The listing builds one solid part. Answer for the finished solid, in the listing's coordinates (mm). Face numbers are marked on the shaded views. A direction names the side the tool comes from. Give positions to 0.01 mm unless a question says otherwise; leave off trailing zeros. Order: outer loops, then holes, each group sorted by start corner. A loop starts at its lowest first (then second) coordinate and runs counter-clockwise, first axis right, second up.
```python
from build123d import *

# Parameters (mm, degrees)
SHANK_PROFILE_12_R           = 6
SHANK_12X27_DEPTH            = 27
SHANK_STEP_9X5_DEPTH         = 29.301943396
SHANK_STEP_9X5_DEPTH_BACK    = 5
SHANK_STEP_PROFILE_9_R       = 6
SHANK_STEP_PROFILE_9_R_2     = 4.5
EYE_PROFILE_20_R             = 10
EYE_PROFILE_20_R_2           = 6
EYE_BOSS_20X25_DEPTH         = 12.5
EYE_START                    = -35
EYE_BORE_PROFILE_R           = 6
EYE_BORE_DEPTH               = 35
CROSS_HOLE_4_DEPTH           = 65.033194649
CROSS_HOLE_4_DEPTH_BACK      = 65.033194649
CROSS_HOLE_PROFILE_4_R       = 2
EYE_BLEND_FILLET_R1_R        = 1
SHANK_STEP_CHAMFER_1X45_SIZE = 1


with BuildPart() as part:
    # Shank Profile Ø12 → Shank Ø12x27 (new body)
    with BuildSketch(Plane.XY):
        Circle(SHANK_PROFILE_12_R)
    extrude(amount=SHANK_12X27_DEPTH)

    # Shank Step Profile Ø9 → Shank Step Ø9x5 (cut, two sides: drawn at the far end of the back side and taken through both)
    with BuildSketch(Plane.XY.offset(27).offset(-SHANK_STEP_9X5_DEPTH_BACK)):
        Circle(SHANK_STEP_PROFILE_9_R)
        Circle(SHANK_STEP_PROFILE_9_R_2, mode=Mode.SUBTRACT)
    extrude(amount=SHANK_STEP_9X5_DEPTH + SHANK_STEP_9X5_DEPTH_BACK, mode=Mode.SUBTRACT)



with BuildPart() as body_2:
    # Eye Profile Ø20 → Eye Boss Ø20x25 (new, symmetric)
    with BuildSketch(Plane(origin=(0, 0, 0), x_dir=(0, 0, -1), z_dir=(1, 0, 0))):
        with Locations((-52, 0)):
            Circle(EYE_PROFILE_20_R)
        with Locations((-52, 0)):
            Circle(EYE_PROFILE_20_R_2, mode=Mode.SUBTRACT)
    extrude(amount=EYE_BOSS_20X25_DEPTH, both=True)


with BuildPart() as part_1:
    add(part.part)

    add(body_2.part)  # Shank To Eye Transition merges body 2
    # Loft End Section 18x20 → Shank To Eye Transition section 0
    with BuildSketch(Plane.XY.offset(52)):
        with BuildLine():
            Line((-9, 10), (9, 10))
            Line((9, 10), (9, -10))
            Line((9, -10), (-9, -10))
            Line((-9, -10), (-9, 10))
        make_face()
    # Loft Start Section 18x15 → Shank To Eye Transition section 1
    with BuildSketch(Plane.XY.offset(27)):
        with BuildLine():
            Line((-9, 7.5), (9, 7.5))
            Line((9, 7.5), (9, -7.5))
            Line((9, -7.5), (-9, -7.5))
            Line((-9, -7.5), (-9, 7.5))
        make_face()
    loft()

    # Eye Bore Profile → Eye Bore (cut)
    with BuildSketch(Plane(origin=(12.5, 0, 0), x_dir=(0, 0, -1), z_dir=(1, 0, 0)).offset(EYE_START)):
        with Locations((-52, 0)):
            Circle(EYE_BORE_PROFILE_R)
    extrude(amount=EYE_BORE_DEPTH, mode=Mode.SUBTRACT)

    # Cross Hole Profile Ø4 → Cross Hole Ø4 (cut, two sides: drawn at the far end of the back side and taken through both)
    with BuildSketch(Plane(origin=(0, 0, 0), x_dir=(0, 0, -1), z_dir=(1, 0, 0)).offset(-CROSS_HOLE_4_DEPTH_BACK)):
        with Locations(Location((-14, 0, 0), (0, 0, 180))):
            Circle(CROSS_HOLE_PROFILE_4_R)
    extrude(amount=CROSS_HOLE_4_DEPTH + CROSS_HOLE_4_DEPTH_BACK, mode=Mode.SUBTRACT)

    # Eye Blend Fillet R1
    eye_blend_fillet_r1_edges = [part_1.edges().sort_by_distance(p)[0] for p in [
        (-9, -6.332377898, 44.260427013),
        (9, 6.332377898, 44.260427013),
        (-6, 0, 0),
    ]]
    fillet(eye_blend_fillet_r1_edges, radius=EYE_BLEND_FILLET_R1_R)

    # Shank Step Chamfer 1x45
    shank_step_chamfer_1x45_edges = [part_1.edges().sort_by_distance(p)[0] for p in [
        (-4.5, 0, 27),
        (-4.5, 0, 22),
    ]]
    chamfer(shank_step_chamfer_1x45_edges, length=SHANK_STEP_CHAMFER_1X45_SIZE)


solid = part_1.part
```
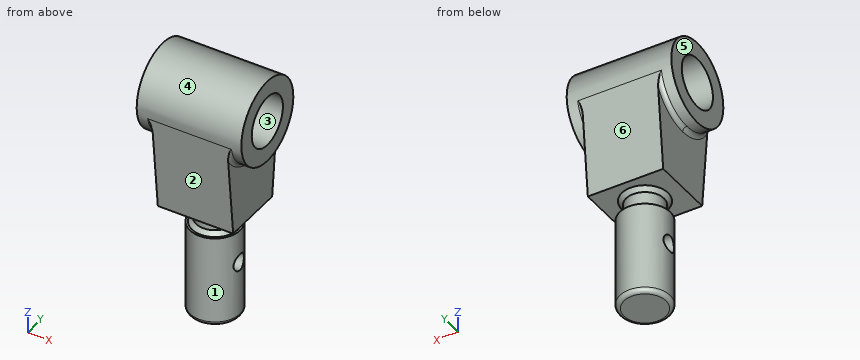
1) Find section D-D (z = 14). Write down the section's boundary in (x, y), then the cut area to 3 significant figures.
Geometry says:
outline: (-5.66, -2) arc R6 ccw to (5.66, -2) - close; (-5.66, 2) - (5.66, 2) arc R6 ccw to start
area: 66.0 mm2
2) Find section A-A (z = 52). Write down the section's boundary in (x, y), then the cut area to 3 significant figures.
Geometry says:
outline: (-12.5, -10) - (12.5, -10) - (12.5, -6) - (-12.5, -6) - close; (-12.5, 6) - (12.5, 6) - (12.5, 10) - (-12.5, 10) - close
area: 200 mm2
3) Straight lines are drawn through the part: probe 1 along Z at (x, y) = (5, -0.75); probe 2 along Z at (x, y) = (-4.5, -1); probe 3 along Y at (x, z) = (-5.25, 52). For each, find the intervals that lie inside material, in ascending order.
Geometry says:
probe 1: z = 0 to 12.15, 15.85 to 22.44, 26.56 to 46.05, 57.95 to 61.97
probe 2: z = 0 to 12.27, 15.73 to 22.89, 26.11 to 46.08, 57.92 to 61.95
probe 3: y = -10 to -6, 6 to 10
4) Given P1, Ø9.5, axis at y = 0, z = 52, coming from the -X side; P2, Ø1.5, axis at x = -4.5, y = 6.5, coming from the -Z side; P3, Ø1.5, axis at x = -5, y = 2.5, coming from the +Z side; P4, Ø3, axis at x = -3.5, z = 13, coming from the -Y side, each flat-ended and moving along its own axis, determine where each tip first touches the part or whether it passes through.
Geometry says:
P1: passes through
P2: stops at z = 27
P3: stops at z = 61.85
P4: stops at y = -5.66
5) A tool of negligible diameter and unlimited length cuts with its end or side. For the marked faces 1 and 2, from which of +Z, -Z, +X, -X, +Y, -Y can it reach the whole face along a straight path? Write none if from no direction.
Geometry says:
face 1: -Z
face 2: -Z, +X, -X, -Y
6) Find section C-C (y = -1). Count the separate pieces of the cut face and the enclosed holes in it, then the cut area to 3 significant figures.
Geometry says:
separate pieces: 3
enclosed holes: 0
area: 738 mm2
7) For a pull along Y with two mould halves and no side action, classify the marked faces 3, 4, 5 and 6 as +Y half, -Y half, draft (parallel to the pull), parting line (faces both ways), or undercut.
Geometry says:
face 3: undercut
face 4: parting line
face 5: draft
face 6: +Y half
8) Find section B-B (x = 0). Write down the section's boundary in (y, z).
Geometry says:
outline: (-9.8, 50.02) - (-7.5, 27) - (-5.5, 27) - (-4.5, 26) - (-4.5, 23) - (-5.5, 22) - (-6, 22) - (-6, 1) arc R1 ccw to (-5, 0) - (5, 0) arc R1 ccw to (6, 1) - (6, 22) - (5.5, 22) - (4.5, 23) - (4.5, 26) - (5.5, 27) - (7.5, 27) - (9.8, 50.02) arc R10 ccw (long way) to start; hole circle Ø12 at (0, 52); hole circle Ø4 at (0, 14)
